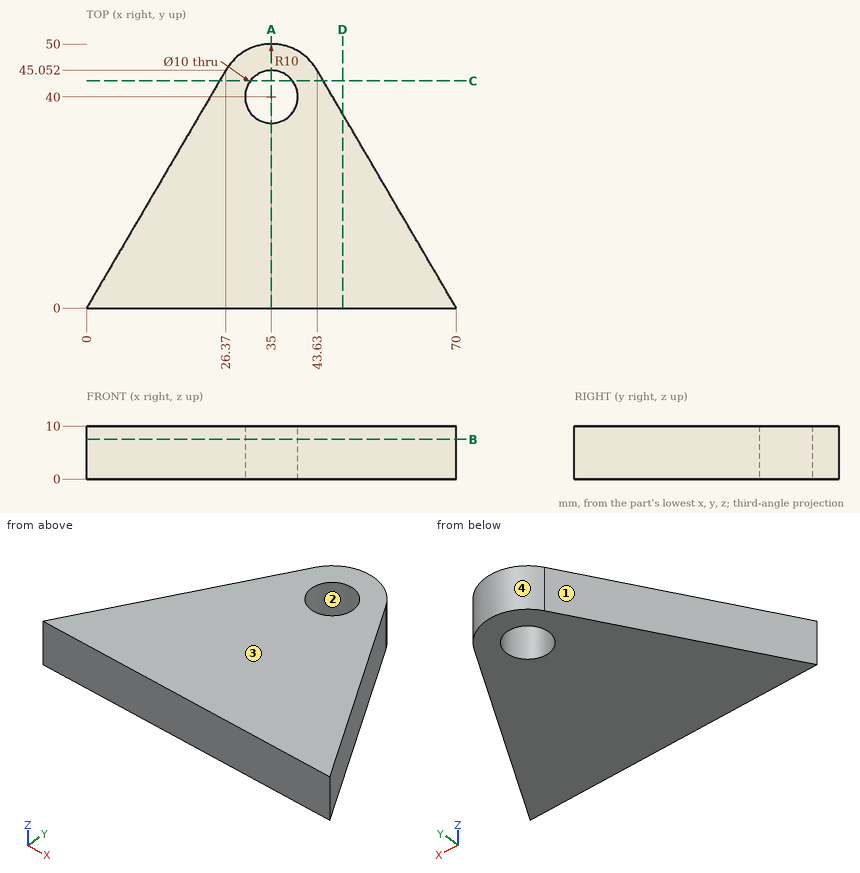
Source: three-view drawing plus pictorial views. Frame: mm from the lowest corner of the part. Coordinates: 2 decimals unless noted, no trailing zeros. Write each loop counter-clockwise with the first axis right and the second up, starting at its lowest first coordinate (ties: lowest second). Pieces come first, ordered by that corner, then holes. Notation, with made-up numbers: (-19.5, 70.25) - (-7.5, 70.25) arc R24 ccw to (-7.5, 104.25) - close; hole circle Ø2 at (25.25, -6.75). An arc over 180 degrees is marked (long way). Answer as a JSON object with one key per item and string values.
Q1. Material intervals for line 1 (Y direction, x = 35, z = 3.25); line 2 (X direction, y = 39, z = 0.5); line 3 (X direction, y = 4, z = 8.25), sorted ascending. Write a range as [from, to].
Ans:
{"line 1": "y = [0, 35], [45, 50]", "line 2": "x = [22.83, 30.1], [39.9, 47.17]", "line 3": "x = [2.34, 67.66]"}
Q2. Draft query along X for the marked faces 1, 2, 3 and 4. Return one class per face: released by +X, released by -X, zero draft, split by the parting line, or undercut.
Ans:
{"face 1": "released by -X", "face 2": "undercut", "face 3": "zero draft", "face 4": "split by the parting line"}
Q3. Section query A-A, the plane x = 35. Output: boundary loops of the cut face in (y, z).
Ans:
{"outline": "(0, 0) - (35, 0) - (35, 10) - (0, 10) - close; (45, 0) - (50, 0) - (50, 10) - (45, 10) - close"}
Q4. First-contact query: pin 1 Ø4 at (y, z) = (38.5, 4) entering from -X (1 decimal); pin 2 Ø3 at (y, z) = (20.5, 3) entering from +X; pin 3 Ø4 at (y, z) = (35.5, 4) entering from -X. Flat tips, straight axial feed; report the tip coordinate or a pass-through.
Ans:
{"pin 1": "stops at x = 21.4", "pin 2": "stops at x = 58.88", "pin 3": "stops at x = 19.61"}
Q5. Section query D-D, the plane x = 48.5. Output: boundary loops of the cut face in (y, z).
Ans:
{"outline": "(0, 0) - (36.73, 0) - (36.73, 10) - (0, 10) - close"}
Q6. Section query B-B, the plane z = 7.5. Output: boundary loops of the cut face in (x, y), plus the area to 3 significant figures.
Ans:
{"outline": "(0, 0) - (70, 0) - (43.63, 45.05) arc R10 ccw to (26.37, 45.05) - close; hole circle Ø10 at (35, 40)", "area": "1,950 mm2"}
Q7. Section query C-C, the plane y = 43. Output: boundary loops of the cut face in (x, z), plus the area to 3 significant figures.
Ans:
{"outline": "(25.17, 0) - (31, 0) - (31, 10) - (25.17, 10) - close; (39, 0) - (44.83, 0) - (44.83, 10) - (39, 10) - close", "area": "117 mm2"}
